from build123d import *

# Parameters (mm, degrees)
SKETCH2_W           = 140
SKETCH2_H           = 200
SKETCH2_R           = 5
BOSS_EXTRUDE1_DEPTH = 10
SKETCH3_R           = 9
SKETCH3_R_2         = 5
BOSS_EXTRUDE2_DEPTH = 25
SKETCH4_R           = 5
BOSS_EXTRUDE3_DEPTH = 1000


with BuildPart() as part:
    # Sketch2 → Boss-Extrude1 (new body)
    with BuildSketch(Plane.XY):
        Rectangle(SKETCH2_W, SKETCH2_H)
        with Locations((-47, 39.5)):
            Circle(SKETCH2_R, mode=Mode.SUBTRACT)
        with Locations((-47, -39.5)):
            Circle(SKETCH2_R, mode=Mode.SUBTRACT)
        with Locations((47, 39.5)):
            Circle(SKETCH2_R, mode=Mode.SUBTRACT)
        with Locations((47, -39.5)):
            Circle(SKETCH2_R, mode=Mode.SUBTRACT)
    extrude(amount=BOSS_EXTRUDE1_DEPTH)

    # Sketch3 → Boss-Extrude2 (add)
    # profile 1 of 4: a face of its own
    with BuildSketch(Plane.XY.offset(10)):
        with Locations((-47, 39.5)):
            Circle(SKETCH3_R)
        with Locations((-47, 39.5)):
            Circle(SKETCH3_R_2, mode=Mode.SUBTRACT)
    # profile 2 of 4: a face of its own
    with BuildSketch(Plane.XY.offset(10)):
        with Locations((47, 39.5)):
            Circle(SKETCH3_R)
        with Locations((47, 39.5)):
            Circle(SKETCH3_R_2, mode=Mode.SUBTRACT)
    # profile 3 of 4: a face of its own
    with BuildSketch(Plane.XY.offset(10)):
        with Locations((47, -39.5)):
            Circle(SKETCH3_R)
        with Locations((47, -39.5)):
            Circle(SKETCH3_R_2, mode=Mode.SUBTRACT)
    # profile 4 of 4: a face of its own
    with BuildSketch(Plane.XY.offset(10)):
        with Locations((-47, -39.5)):
            Circle(SKETCH3_R)
        with Locations((-47, -39.5)):
            Circle(SKETCH3_R_2, mode=Mode.SUBTRACT)
    extrude(amount=BOSS_EXTRUDE2_DEPTH)

    # Sketch4 → Boss-Extrude3 (add)
    with BuildSketch(Plane(origin=(0, 0, 0), x_dir=(-1, 0, 0), z_dir=(0, 0, -1))):
        with Locations((-47, 39.5)):
            Circle(SKETCH4_R)
        with Locations((47, 39.5)):
            Circle(SKETCH4_R)
        with Locations((47, -39.5)):
            Circle(SKETCH4_R)
        with Locations((-47, -39.5)):
            Circle(SKETCH4_R)
    extrude(amount=-BOSS_EXTRUDE3_DEPTH)


solid = part.part
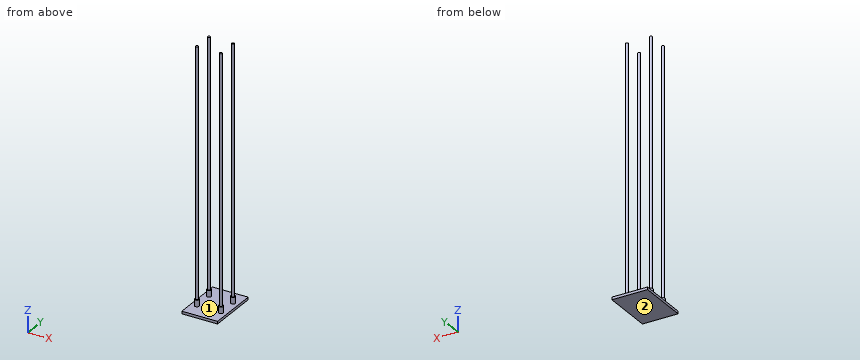
Read the model definition and answer for the solid it produces. Units are mm, in the model's axes. Face numbers are marked on the shaded views. A direction names the side the tool comes from. Round coordinates to 2 decimals unless told otherwise and drop trailing zeros. Write each loop counter-clockwise with the first axis right and the second up, starting at its lowest first coordinate (ties: lowest second). Pieces come first, ordered by that corner, then holes. Notation, with made-up numbers: (13.25, -13) - (27.25, -13) arc R14 cw to (27.25, -3) - close; hole circle Ø11 at (43, 22). An arc over 180 degrees is marked (long way). One line per question, with ' | ' between items. Start each with the question number.
1. Section C-C (x = -8.5) is taken. Determine the outline of the cut face in (y, z).
2. Each of these flat-tipped pins is pushed along its axis until it touches: pin 1 (12 mm diameter, centred on x = 30, y = 33, fed in from -Z); pin 2 (10 mm diameter, centred on x = 51.5, z = 710.5, fed in from -Y); pin 3 (1 mm diameter, centred on x = -50.5, z = 393, fed in from +Y); pin 4 (6 mm diameter, centred on x = 42.5, z = 194.5, fed in from -Y). Where does it stop, or does it pass through?
3. Section A-A (z = 102) is taken. Determine the outline of the cut face in (x, y).
4. For the marked faces 1 and 2, determine the directions among +Z, -Z, +X, -X, +Y, -Y from which every point of the face is accessible in a straight line to the end or side of a thin tool.
5. Find the intervals of material crossed by probe 1 along Z at (x, y) = (30.5, 4.5); probe 2 along X at (y, z) = (36, 847); probe 3 along Y at (x, z) = (-48, 506), in increasing order. Write a range as [from, to].
6. Section B-B (y = 57.5) is taken. Determine the outline of the cut face in (x, z), and give its area (3 significant figures).
Filled in:
1) outline: (-100, 0) - (100, 0) - (100, 10) - (-100, 10) - close
2) pin 1: z = 0 | pin 2: y = -44.5 | pin 3: y = 43.5 | pin 4: y = -44.27
3) outline: circle Ø10 at (-47, -39.5); circle Ø10 at (-47, 39.5); circle Ø10 at (47, -39.5); circle Ø10 at (47, 39.5)
4) face 1: +Z | face 2: -Z, +X, -X, +Y, -Y
5) probe 1: [0, 10] | probe 2: [-50.57, -43.43], [43.43, 50.57] | probe 3: [-44.4, -34.6], [34.6, 44.4]
6) outline: (-70, 0) - (70, 0) - (70, 10) - (-70, 10) - close | area: 1,400 mm²
